```python
from build123d import *

# Parameters (mm, degrees)
BOSS_EXTRUDE1_DEPTH = 4


with BuildPart() as part:
    # Sketch1 → Boss-Extrude1 (new body)
    with BuildSketch(Plane.XY):
        Polygon((3, 0), (35, 0), (35, 40), (0, 40), (0, 5.997826072), (3, 5.997826072), align=None)
        with BuildLine():
            Line((9.5, 29), (9.5, 19))
            ThreePointArc((9.5, 19), (17.5, 11), (25.5, 19))
            Line((25.5, 19), (25.5, 29))
            ThreePointArc((25.5, 29), (17.5, 37), (9.5, 29))
        make_face(mode=Mode.SUBTRACT)
    extrude(amount=BOSS_EXTRUDE1_DEPTH)


solid = part.part
```
Design review of the part built by this model. Coordinates are the model's own, in mm. A direction names the side the tool comes from. Round coordinates to 2 decimals unless told otherwise and drop trailing zeros. Write each loop counter-clockwise with the first axis right and the second up, starting at its lowest first coordinate (ties: lowest second). Pieces come first, ordered by that corner, then holes. Notation, with made-up numbers: (25.25, 44) -> (69.25, 44) arc R23 cw to (69.25, 78) -> close; hole circle Ø5 at (19, 70). An arc over 180 degrees is marked (long way). Answer in a Markdown table with one row per item.
Q1. Take a section at B-B, the plane x = 17.5. State the section outline as (y, z) points.
The answers:
| item | result |
|---|---|
| outline | (0, 0) -> (11, 0) -> (11, 4) -> (0, 4) -> close; (37, 0) -> (40, 0) -> (40, 4) -> (37, 4) -> close |
Q2. For faces 1 (the face through (1, 5.998, 2)), 2 (the face through (25.5, 24, 2)), 3 (the face through (9, 20, 4)), list the 3-axis set-ups (+Z, -Z, +X, -X, +Y, -Y) from which the entire face can be reached by the end or side of a thin tool; tool diameter is ignored.
The answers:
| item | result |
|---|---|
| face 1 | +Z, -Z, -X, -Y |
| face 2 | +Z, -Z |
| face 3 | +Z, +X, -X, +Y, -Y |
Q3. To check wall thickness, follow L1, parallel to X at y = 24.5, z = 2.25; L2, parallel to X at y = 5, z = 3.25; L3, parallel to Y at x = 17, z = 3.5. State the ranges of each line that lie inside material, in increasing order. Write a range as [from, to].
The answers:
| item | result |
|---|---|
| L1 | [0, 9.5], [25.5, 35] |
| L2 | [3, 35] |
| L3 | [0, 11.02], [36.98, 40] |
Q4. Clearance check with a flat-ended pin moving along its axis: pin 1 Ø0.9 at (x, z) = (1.5, 2.5) entering from -Y. State where the tip first meets the part, or that it passes through.
The answers:
| item | result |
|---|---|
| pin 1 | y = 6 |
Q5. Take a section at A-A, the plane z = 2.75. State the section outline as (x, y) points, then the cut area to 3 significant figures.
The answers:
| item | result |
|---|---|
| outline | (0, 6) -> (3, 6) -> (3, 0) -> (35, 0) -> (35, 40) -> (0, 40) -> close; hole (9.5, 19) arc R8 ccw to (25.5, 19) -> (25.5, 29) arc R8 ccw to (9.5, 29) -> close |
| area | 1,020 mm² |
Q6. Take a section at C-C, the plane y = 35.5. State the section outline as (x, z) points, then the cut area to 3 significant figures.
The answers:
| item | result |
|---|---|
| outline | (0, 0) -> (12.84, 0) -> (12.84, 4) -> (0, 4) -> close; (22.16, 0) -> (35, 0) -> (35, 4) -> (22.16, 4) -> close |
| area | 103 mm² |
